```python
from build123d import *

# Parameters (mm, degrees)
SKETCH1_W                                            = 168
SKETCH1_H                                            = 135
BOSS_EXTRUDE1_DEPTH                                  = 15
HOLE_SIZE_PER_SOCKET_HEAD_CAP_SCREW_TYPE_D           = 9
HOLE_SIZE_PER_SOCKET_HEAD_CAP_SCREW_TYPE_CBORE_D     = 15
HOLE_SIZE_PER_SOCKET_HEAD_CAP_SCREW_TYPE_CBORE_DEPTH = 9
CHAMFER1_SIZE                                        = 1


with BuildPart() as part:
    # Sketch1 → Boss-Extrude1 (new body)
    with BuildSketch(Plane.XY):
        Rectangle(SKETCH1_W, SKETCH1_H)
    extrude(amount=BOSS_EXTRUDE1_DEPTH)

    # Hole size per socket head cap screw type1 (through all)
    with Locations(Plane.XY.offset(15)):
        with Locations((-74, 25), (-74, -25), (74, -25), (74, 25)):
            CounterBoreHole(HOLE_SIZE_PER_SOCKET_HEAD_CAP_SCREW_TYPE_D / 2, HOLE_SIZE_PER_SOCKET_HEAD_CAP_SCREW_TYPE_CBORE_D / 2, HOLE_SIZE_PER_SOCKET_HEAD_CAP_SCREW_TYPE_CBORE_DEPTH)

    # Chamfer1
    chamfer1_edges = [part.edges().sort_by_distance(p)[0] for p in [
        (84, -67.5, 7.5),
        (-84, -67.5, 7.5),
        (-84, 67.5, 7.5),
        (84, 67.5, 7.5),
    ]]
    chamfer(chamfer1_edges, length=CHAMFER1_SIZE)


solid = part.part
```
The listing builds one solid part. Answer for the finished solid, in the listing's coordinates (mm). A direction names the side the tool comes from. Round coordinates to 2 decimals unless told otherwise and drop trailing zeros. Loops run counter-clockwise (first coordinate to the right, second up) from the corner with the lowest first, then second, coordinate; pieces in that order, holes last.
1) A cutting plane is placed at A-A on x = 74. Determine the outline of the cut face in (y, z).
Outcome:
outline: (-67.5, 0) - (-29.5, 0) - (-29.5, 6) - (-32.5, 6) - (-32.5, 15) - (-67.5, 15) - close; (-20.5, 0) - (20.5, 0) - (20.5, 6) - (17.5, 6) - (17.5, 15) - (-17.5, 15) - (-17.5, 6) - (-20.5, 6) - close; (29.5, 0) - (67.5, 0) - (67.5, 15) - (32.5, 15) - (32.5, 6) - (29.5, 6) - close
2) A cutting plane is placed at C-C on z = 9.5. Determine the outline of the cut face in (x, y).
Outcome:
outline: (-84, -66.5) - (-83, -67.5) - (83, -67.5) - (84, -66.5) - (84, 66.5) - (83, 67.5) - (-83, 67.5) - (-84, 66.5) - close; hole circle Ø15 at (-74, -25); hole circle Ø15 at (-74, 25); hole circle Ø15 at (74, -25); hole circle Ø15 at (74, 25)
3) Consider line 1 (Y direction, x = 74, z = 2.35); line 2 (X direction, y = -31, z = 10.75); line 3 (X direction, y = -27, z = 1.75). Determine where each line is inside the solid, lowest interval first.
Outcome:
line 1: y = -67.5 to -29.5, -20.5 to 20.5, 29.5 to 67.5
line 2: x = -84 to -78.5, -69.5 to 69.5, 78.5 to 84
line 3: x = -84 to -78.03, -69.97 to 69.97, 78.03 to 84
4) For faces 4 (the face through (-79.5, 30.1, 10.6)), 5 (the face through (-76.419, 28.794, 2.958)), determine the directions among +Z, -Z, +X, -X, +Y, -Y from which every point of the face is accessible in a straight line to the end or side of a thin tool.
Outcome:
face 4: +Z
face 5: +Z, -Z
5) Given P1, Ø14.5, axis at x = -74, y = -25, coming from the +Z side; P2, Ø24, axis at x = 74, y = 25, coming from the +Z side, each flat-ended and moving along its own axis, determine where each tip first touches the part or whether it passes through.
Outcome:
P1: stops at z = 6
P2: stops at z = 15
6) For a pull along Y with two mould halves and no side action, classify faces 1 (the face through (68.5, 30.1, 10.6)), 2 (the face through (-1, 1, 15)), 3 (the face through (-1, 67.5, 7)) as released by +Y, released by -Y, zero draft, split by the parting line, or undercut.
Outcome:
face 1: undercut
face 2: zero draft
face 3: released by +Y
7) A cutting plane is placed at B-B on y = 25. Determine the outline of the cut face in (x, z), plus the area to 3 significant figures.
Outcome:
outline: (-84, 0) - (-78.5, 0) - (-78.5, 6) - (-81.5, 6) - (-81.5, 15) - (-84, 15) - close; (-69.5, 0) - (69.5, 0) - (69.5, 6) - (66.5, 6) - (66.5, 15) - (-66.5, 15) - (-66.5, 6) - (-69.5, 6) - close; (78.5, 0) - (84, 0) - (84, 15) - (81.5, 15) - (81.5, 6) - (78.5, 6) - close
area: 2,140 mm2
